Check sheet for the drawn part. Datum: minimum x, y, z corner. Units: mm. Give positions to 0.01 mm unless a question says otherwise; leave off trailing zeros. Write each loop counter-clockwise with the first axis right and the second up, starting at its lowest first coordinate (ties: lowest second). Pieces come first, ordered by that corner, then holes. Notation, with made-up numbers: (36.25, 19) - (63.25, 19) arc R35 ccw to (63.25, 51) - close; hole circle Ø1 at (-37, 41.5). An arc over 180 degrees is marked (long way). Use a Markdown table: item, result.
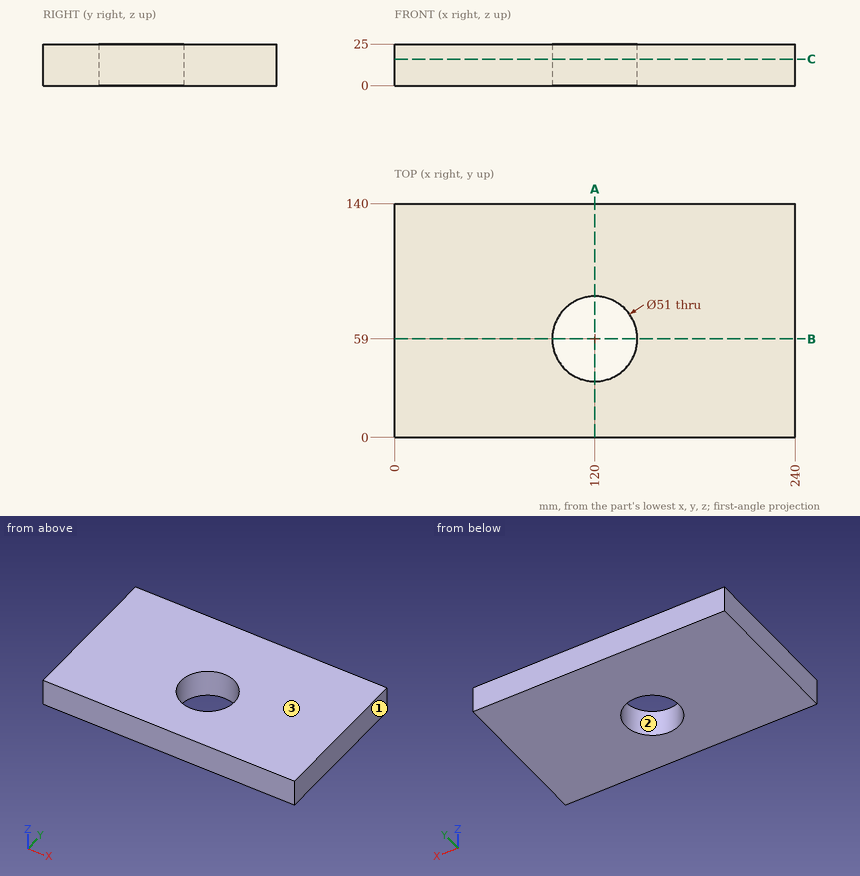
1) Section check A-A on x = 120. Record the boundary of the cut face in (y, z).
Working result:
| item | result |
|---|---|
| outline | (0, 0) - (33.5, 0) - (33.5, 25) - (0, 25) - close; (84.5, 0) - (140, 0) - (140, 25) - (84.5, 25) - close |
2) Material ranges on L1, parallel to Y at x = 120, z = 10.5; L2, parallel to X at y = 75, z = 11.5; L3, parallel to Y at x = 127, z = 6, recorded low to high. Write a range as from..to.
Working result:
| item | result |
|---|---|
| L1 | y = 0..33.5, 84.5..140 |
| L2 | x = 0..100.14, 139.86..240 |
| L3 | y = 0..34.48, 83.52..140 |
3) Section check B-B on y = 59. Record the boundary of the cut face in (x, z), then the cut area to 4 significant figures.
Working result:
| item | result |
|---|---|
| outline | (0, 0) - (94.5, 0) - (94.5, 25) - (0, 25) - close; (145.5, 0) - (240, 0) - (240, 25) - (145.5, 25) - close |
| area | 4,725 mm² |
4) Section check C-C on z = 16. Record the boundary of the cut face in (x, y).
Working result:
| item | result |
|---|---|
| outline | (0, 0) - (240, 0) - (240, 140) - (0, 140) - close; hole circle Ø51 at (120, 59) |
5) Mould release check, pull along X, two halves, no side actions. Record for the marked faces 1, 2 and 3: pulls with the +X half, pulls with the -X half, needs draft (parallel to the pull), parting line crosses it, or undercut.
Working result:
| item | result |
|---|---|
| face 1 | pulls with the +X half |
| face 2 | undercut |
| face 3 | needs draft |
